from build123d import *

# Parameters (mm, degrees)
BOSS_EXTRUDE1_DEPTH            = 74
SKETCH2_W                      = 64
SKETCH2_H                      = 74
BOSS_EXTRUDE2_DEPTH            = 14
SKETCH3_W                      = 64
SKETCH3_H                      = 78
BOSS_EXTRUDE3_DEPTH            = 4
CUT_EXTRUDE1_DEPTH             = 70
SKETCH5_W                      = 78
SKETCH5_H                      = 78
BOSS_EXTRUDE4_DEPTH            = 14
CUT_EXTRUDE2_REACH             = 115.771
SKETCH7_W                      = 64
SKETCH7_H                      = 70
CUT_EXTRUDE3_REACH             = 124.581
SKETCH9_W                      = 70
SKETCH9_H                      = 70
CUT_EXTRUDE4_DEPTH             = 110.936081615
CUT_EXTRUDE5_DEPTH             = 123.581337469
CUT_EXTRUDE6_DEPTH             = 119.860244595
CUT_EXTRUDE7_DEPTH             = 119.860244595
CUT_EXTRUDE8_DEPTH             = 128.31922202
F_8_5_8_5_DIAMETER_HOLE1_D     = 8.5
F_8_5_8_5_DIAMETER_HOLE1_DEPTH = 78
F_8_5_8_5_DIAMETER_HOLE2_D     = 8.5
F_8_5_8_5_DIAMETER_HOLE2_DEPTH = 78
CHAMFER1_SIZE                  = 4


with BuildPart() as part:
    # Sketch1 → Boss-Extrude1 (new body)
    with BuildSketch(Plane(origin=(0, 78, 0), x_dir=(1, 0, 0), z_dir=(0, 1, 0))):
        Polygon((-19.730848831, -49.578174681), (37.269151169, -49.578174681), (-19.730848831, 7.421825319), align=None)
    extrude(amount=-BOSS_EXTRUDE1_DEPTH)

    # Sketch2 → Boss-Extrude2 (add)
    with BuildSketch(Plane.XY.offset(49.578174681)):
        with Locations((12.269151169, 41)):
            Rectangle(SKETCH2_W, SKETCH2_H)
    extrude(amount=BOSS_EXTRUDE2_DEPTH)

    # Sketch3 → Boss-Extrude3 (add)
    with BuildSketch(Plane.XZ.offset(-4)):
        with Locations((12.269151169, 24.578174681)):
            Rectangle(SKETCH3_W, SKETCH3_H)
    extrude(amount=BOSS_EXTRUDE3_DEPTH)

    # Sketch4 → Cut-Extrude1 (cut)
    with BuildSketch(Plane.XZ.offset(-4)):
        Polygon((-19.730848831, -7.421825319), (37.269151169, 49.578174681), (-19.730848831, 49.578174681), align=None)
    extrude(amount=-CUT_EXTRUDE1_DEPTH, mode=Mode.SUBTRACT)

    # Sketch5 → Boss-Extrude4 (add)
    with BuildSketch(Plane.ZY.offset(19.730848831)):
        with Locations((24.578174681, 39)):
            Rectangle(SKETCH5_W, SKETCH5_H)
    extrude(amount=BOSS_EXTRUDE4_DEPTH)

    # Sketch7 → Cut-Extrude2 (cut, up to next)
    with BuildSketch(Plane.XY.offset(55.578174681), mode=Mode.PRIVATE) as cut_extrude2_sk1:
        with Locations((12.269151169, 39)):
            Rectangle(SKETCH7_W, SKETCH7_H)
    cut_extrude2_tool1 = extrude(cut_extrude2_sk1.sketch, amount=-CUT_EXTRUDE2_REACH, mode=Mode.PRIVATE) & part.part
    add(cut_extrude2_tool1.solids().sort_by_distance((12.269151, 39, 55.578175))[0], mode=Mode.SUBTRACT)

    # Sketch9 → Cut-Extrude3 (cut, up to next)
    with BuildSketch(Plane(origin=(-25.730848831, 0, 0), x_dir=(0, -1, 0), z_dir=(-1, 0, 0)), mode=Mode.PRIVATE) as cut_extrude3_sk1:
        with Locations((-39, 20.578174681)):
            Rectangle(SKETCH9_W, SKETCH9_H)
    cut_extrude3_tool1 = extrude(cut_extrude3_sk1.sketch, amount=-CUT_EXTRUDE3_REACH, mode=Mode.PRIVATE) & part.part
    add(cut_extrude3_tool1.solids().sort_by_distance((-25.730849, 39, 20.578175))[0], mode=Mode.SUBTRACT)

    # Sketch10 → Cut-Extrude4 (cut, through all)
    with BuildSketch(Plane.XZ):
        Polygon((44.269151169, 49.578174681), (37.269151169, 49.578174681), (-19.730848831, -7.421825319), (-19.730848831, -14.421825319), (44.269151169, -14.421825319), align=None)
    extrude(amount=-CUT_EXTRUDE4_DEPTH, mode=Mode.SUBTRACT)

    # Sketch11 → Cut-Extrude5 (cut, through all)
    with BuildSketch(Plane(origin=(-25.730848831, 0, 0), x_dir=(0, 0, -1), z_dir=(1, 0, 0))):
        with BuildLine():
            Line((-23.578174681, 24), (-40.578174681, 24))
            ThreePointArc((-40.578174681, 24), (-45.578174681, 19), (-40.578174681, 14))
            Line((-40.578174681, 14), (-23.578174681, 14))
            ThreePointArc((-23.578174681, 14), (-18.578174681, 19), (-23.578174681, 24))
        make_face()
    extrude(amount=-CUT_EXTRUDE5_DEPTH, mode=Mode.SUBTRACT)

    # Sketch12 → Cut-Extrude6 (cut, through all)
    with BuildSketch(Plane.XY.offset(63.578174681)):
        with BuildLine():
            Line((6.269151169, 64), (-10.730848831, 64))
            ThreePointArc((-10.730848831, 64), (-15.730848831, 59), (-10.730848831, 54))
            Line((-10.730848831, 54), (6.269151169, 54))
            ThreePointArc((6.269151169, 54), (11.269151169, 59), (6.269151169, 64))
        make_face()
    extrude(amount=-CUT_EXTRUDE6_DEPTH, mode=Mode.SUBTRACT)

    # Sketch13 → Cut-Extrude7 (cut, through all)
    with BuildSketch(Plane.XY.offset(63.578174681)):
        with BuildLine():
            Line((6.269151169, 24), (-10.730848831, 24))
            ThreePointArc((-10.730848831, 24), (-15.730848831, 19), (-10.730848831, 14))
            Line((-10.730848831, 14), (6.269151169, 14))
            ThreePointArc((6.269151169, 14), (11.269151169, 19), (6.269151169, 24))
        make_face()
    extrude(amount=-CUT_EXTRUDE7_DEPTH, mode=Mode.SUBTRACT)

    # Sketch14 → Cut-Extrude8 (cut, through all)
    with BuildSketch(Plane.ZY.offset(33.730848831)):
        with BuildLine():
            Line((23.078174681, 54), (40.078174681, 54))
            ThreePointArc((40.078174681, 54), (45.078174681, 59), (40.078174681, 64))
            Line((40.078174681, 64), (23.078174681, 64))
            ThreePointArc((23.078174681, 64), (18.078174681, 59), (23.078174681, 54))
        make_face()
    extrude(amount=-CUT_EXTRUDE8_DEPTH, mode=Mode.SUBTRACT)

    # Ø8.5 (8.5) Diameter Hole1
    with Locations(Plane.ZY.offset(33.730848831)):
        with Locations((1.578174681, 59), (1.578174681, 19)):
            Hole(F_8_5_8_5_DIAMETER_HOLE1_D / 2, depth=F_8_5_8_5_DIAMETER_HOLE1_DEPTH)

    # Ø8.5 (8.5) Diameter Hole2
    with Locations(Plane.XY.offset(63.578174681)):
        with Locations((28.269151169, 19), (28.269151169, 59)):
            Hole(F_8_5_8_5_DIAMETER_HOLE2_D / 2, depth=F_8_5_8_5_DIAMETER_HOLE2_DEPTH)

    # Chamfer1
    chamfer1_edges = [part.edges().sort_by_distance(p)[0] for p in [
        (-33.730848831, 39, 63.578174681),
    ]]
    chamfer(chamfer1_edges, length=CHAMFER1_SIZE)


solid = part.part
Here's how the part is built. I have some questions about the finished solid (model axes, mm). A direction names the side the tool comes from. Coordinates: 2 decimals unless noted, no trailing zeros. Loops run counter-clockwise (first coordinate to the right, second up) from the corner with the lowest first, then second, coordinate; pieces in that order, holes last.
1. For P1, Ø4, axis at x = 3, y = 37, coming from the -Z side; P2, Ø4.5, axis at y = 76.5, z = -10, coming from the +X side; P3, Ø4, axis at y = 13, z = 6.5, coming from the +X side; P4, Ø7, axis at y = 19, z = 1.58, coming from the +X side, each with a flat end and sliding along its axis, tell me the tip position at first contact or that it passes through.
2. Imagine slicing it at C-C, the plane x = 10. Please give me the cut outline in (y, z).
3. I need wall thicknesses on L1, parallel to Y at x = 40, z = 51; L2, parallel to Z at x = -15, y = 35; L3, parallel to X at y = 9, z = 9. Which ranges of each line are inside material? Lowest first, please.
4. For faces 4 (the flat face through (-2, 14, 60)), 5 (the flat face through (-19.731, 76, -11)), 6 (the flat face through (-7, 74, 36)), 7 (the flat face through (-30, 64, 32)), which set-ups out of +Z, -Z, +X, -X, +Y, -Y let a thin tool reach every point of the face, with its end or its side?
5. Imagine slicing it at A-A, the plane z = 2. Please give me the cut outline in (x, y).
6. Imagine slicing it at D-D, the plane y = 45. Please give me the cut outline in (x, z).
7. Imagine slicing it at B-B, the plane y = 19. Please give me the cut outline in (x, z), and give its area (3 significant figures).
8. If we mould it in two halves opening along Y, with no side actions, what happens to faces 1 (the flat face through (9.17, 1.97, 21.48)), 2 (the cylindrical face through (-29.787, 58.89, 45.077)), 3 (the flat face through (-3, 0, 33))? For each: pulls with the +Y half, pulls with the -Y half, needs draft (parallel to the pull), parting line crosses it, or undercut.
Taken from the geometry:
1. P1: stops at z = 55.58
1. P2: stops at x = -19.73
1. P3: stops at x = -25.73
1. P4: passes through
2. outline: (0, 22.31) - (4, 22.31) - (4, 55.58) - (15.67, 55.58) - (15.67, 63.58) - (0, 63.58) - close; (22.33, 55.58) - (55.67, 55.58) - (55.67, 63.58) - (22.33, 63.58) - close; (62.33, 55.58) - (74, 55.58) - (74, 22.31) - (78, 22.31) - (78, 63.58) - (62.33, 63.58) - close
3. L1: y = 0 to 4, 74 to 78
3. L2: z = 55.58 to 63.58
3. L3: x = -33.73 to -25.73
4. face 4: +Z, -Z
4. face 5: -Z, +X, +Y, -Y
4. face 6: -Z, +X
4. face 7: +X, -X
5. outline: (-33.73, 0) - (-10.31, 0) - (-10.31, 4) - (-25.73, 4) - (-25.73, 14.77) - (-33.73, 14.77) - close; (-33.73, 23.23) - (-25.73, 23.23) - (-25.73, 54.77) - (-33.73, 54.77) - close; (-33.73, 63.23) - (-25.73, 63.23) - (-25.73, 74) - (-10.31, 74) - (-10.31, 78) - (-33.73, 78) - close
6. outline: (-33.73, -14.42) - (-25.73, -14.42) - (-25.73, 55.58) - (44.27, 55.58) - (44.27, 63.58) - (-29.73, 63.58) - (-33.73, 59.58) - close
7. outline: (-33.73, -14.42) - (-25.73, -14.42) - (-25.73, -2.67) - (-33.73, -2.67) - close; (-33.73, 5.83) - (-25.73, 5.83) - (-25.73, 18.58) - (-33.73, 18.58) - close; (-33.73, 45.58) - (-25.73, 45.58) - (-25.73, 55.58) - (-15.73, 55.58) - (-15.73, 63.58) - (-29.73, 63.58) - (-33.73, 59.58) - close; (11.27, 55.58) - (24.02, 55.58) - (24.02, 63.58) - (11.27, 63.58) - close; (32.52, 55.58) - (44.27, 55.58) - (44.27, 63.58) - (32.52, 63.58) - close
7. area: 608 mm2
8. face 1: needs draft
8. face 2: undercut
8. face 3: pulls with the -Y half
